```python
from build123d import *

# Parameters (mm, degrees)
SKETCH1_R           = 22.5
SKETCH1_R_2         = 14.75
BOSS_EXTRUDE1_DEPTH = 25
SKETCH2_R           = 17.5
SKETCH2_R_2         = 14.75
BOSS_EXTRUDE2_DEPTH = 5
CHAMFER2_SIZE       = 1


with BuildPart() as part:
    # Sketch1 → Boss-Extrude1 (new body)
    with BuildSketch(Plane.XY):
        Circle(SKETCH1_R)
        Circle(SKETCH1_R_2, mode=Mode.SUBTRACT)
    extrude(amount=BOSS_EXTRUDE1_DEPTH)

    # Sketch2 → Boss-Extrude2 (add)
    with BuildSketch(Plane.XY.offset(25)):
        Circle(SKETCH2_R)
        Circle(SKETCH2_R_2, mode=Mode.SUBTRACT)
    extrude(amount=BOSS_EXTRUDE2_DEPTH)

    # Chamfer2
    chamfer2_edges = [part.edges().sort_by_distance(p)[0] for p in [
        (-17.5, 0, 30),
        (-22.5, 0, 0),
        (-22.5, 0, 25),
    ]]
    chamfer(chamfer2_edges, length=CHAMFER2_SIZE)


solid = part.part
```
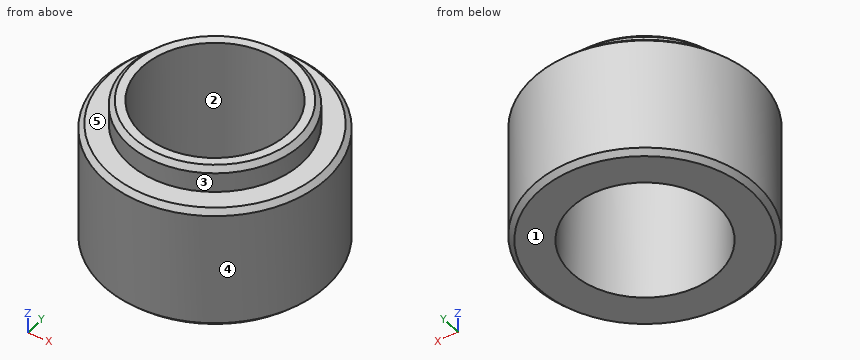
The model under review builds one solid part; all positions refer to its coordinate system, in mm. Face numbers are marked on the shaded views. A direction names the side the tool comes from. Round coordinates to 2 decimals unless told otherwise and drop trailing zeros. Loops run counter-clockwise (first coordinate to the right, second up) from the corner with the lowest first, then second, coordinate; pieces in that order, holes last.
Item 1: Mouldability with a two-part tool opening along Y and no side actions: class the marked faces 1, 2 and 3 as released by +Y, released by -Y, zero draft, split by the parting line, or undercut.
Determined:
face 1: zero draft
face 2: undercut
face 3: split by the parting line
Item 2: Take a section at C-C (z = 20.5). Write out the cut boundary in (x, y).
Determined:
outline: circle Ø45 at (0, 0); hole circle Ø29.5 at (0, 0)
Item 3: For line 1 (Y direction, x = 0, z = 13); line 2 (X direction, y = -0.5, z = 11.5); line 3 (Z direction, x = -5.5, y = 20), list the stretches that pass through material, from the lowest coordinate up.
Determined:
line 1: y = -22.5 to -14.75, 14.75 to 22.5
line 2: x = -22.49 to -14.74, 14.74 to 22.49
line 3: z = 0 to 25
Item 4: Clearance check with flat-ended pins moving along their axes: pin 1 Ø8 at (y, z) = (4.5, 8.5) entering from -X; pin 2 Ø1 at (y, z) = (-7, 18.5) entering from +X; pin 3 Ø1.5 at (x, z) = (17.5, 20.5) entering from +Y. State where each tip first meets the part, or that it passes through.
Determined:
pin 1: stops at x = -22.49
pin 2: stops at x = 21.54
pin 3: stops at y = 15.02
Item 5: Take a section at A-A (x = 0). Write out the cut boundary in (y, z).
Determined:
outline: (-22.5, 1) - (-21.5, 0) - (-14.75, 0) - (-14.75, 30) - (-16.5, 30) - (-17.5, 29) - (-17.5, 25) - (-21.5, 25) - (-22.5, 24) - close; (14.75, 0) - (21.5, 0) - (22.5, 1) - (22.5, 24) - (21.5, 25) - (17.5, 25) - (17.5, 29) - (16.5, 30) - (14.75, 30) - close
Item 6: For the marked faces 4 and 5, list the 3-axis set-ups (+Z, -Z, +X, -X, +Y, -Y) from which the entire face can be reached by the end or side of a thin tool; tool diameter is ignored.
Determined:
face 4: +Z, -Z
face 5: +Z
